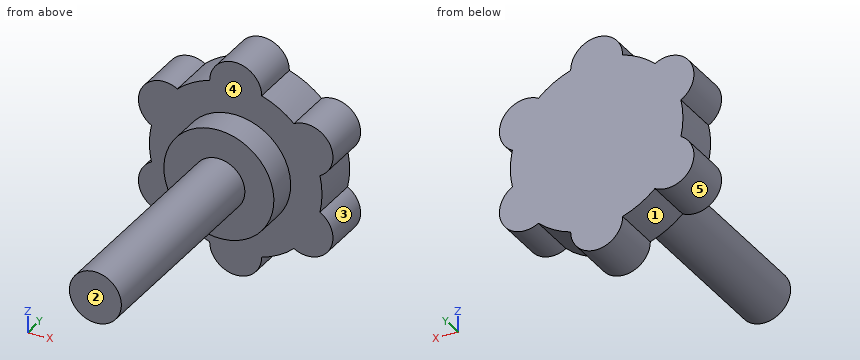
```python
from build123d import *

# Parameters (mm, degrees)
BOSS_EXTRUDE1_DEPTH = 5.6
SKETCH2_R           = 6.35
BOSS_EXTRUDE2_DEPTH = 3.4
SKETCH3_R           = 3
BOSS_EXTRUDE3_DEPTH = 25


with BuildPart() as part:
    # Sketch1 → Boss-Extrude1 (new body)
    with BuildSketch(Plane(origin=(0, 0, 0), x_dir=(1, 0, 0), z_dir=(0, 1, 0))):
        with BuildLine():
            Line((-9.72424134, -2.15192377), (-9.725740285, -2.152789186))
            ThreePointArc((-9.725740285, -2.152789186), (-10.823817926, -6.250865027), (-6.725742085, -7.348942669))
            Line((-6.725742085, -7.348942669), (-6.723420775, -7.34760246))
            ThreePointArc((-6.723420775, -7.34760246), (-4.978167749, -8.626268935), (-2.998, -9.497952231))
            Line((-2.998, -9.497952231), (-2.998, -9.5))
            ThreePointArc((-2.998, -9.5), (0.002000003, -12.499999996), (3.002, -9.499999993))
            Line((3.002, -9.499999993), (3.002, -9.497636397))
            ThreePointArc((3.002, -9.497636397), (4.982303032, -8.625613539), (6.727581168, -7.346540363))
            Line((6.727581168, -7.346540363), (6.728741336, -7.347210186))
            ThreePointArc((6.728741336, -7.347210186), (10.826817547, -6.249133975), (9.728741336, -2.151057763))
            Line((9.728741336, -2.151057763), (9.727581168, -2.15038794))
            ThreePointArc((9.727581168, -2.15038794), (9.962651964, 0.001128196), (9.727467916, 2.152631955))
            ThreePointArc((9.727467916, 2.152631955), (10.825817547, 6.250866025), (6.727194396, 7.348626461))
            ThreePointArc((6.727194396, 7.348626461), (4.981167779, 8.628000969), (3, 9.5))
            ThreePointArc((3, 9.5), (2e-09, 12.5), (-3, 9.499052498))
            ThreePointArc((-3, 9.499052498), (-4.980665222, 8.626558938), (-6.726128008, 7.346856081))
            ThreePointArc((-6.726128008, 7.346856081), (-10.824817547, 6.249133975), (-9.726741336, 2.151057764))
            Line((-9.726741336, 2.151057764), (-9.725033927, 2.150071991))
            ThreePointArc((-9.725033927, 2.150071991), (-9.959651798, -0.000969188), (-9.72424134, -2.15192377))
        make_face()
    extrude(amount=BOSS_EXTRUDE1_DEPTH)

    # Sketch2 → Boss-Extrude2 (add)
    with BuildSketch(Plane.XZ):
        with Locations(Location((0, 0, 0), (0, 0, 90))):
            Circle(SKETCH2_R)
    extrude(amount=BOSS_EXTRUDE2_DEPTH)

    # Sketch3 → Boss-Extrude3 (add)
    with BuildSketch(Plane.XZ.offset(3.4)):
        with Locations(Location((0, 0, 0), (0, 0, 270))):
            Circle(SKETCH3_R)
    extrude(amount=BOSS_EXTRUDE3_DEPTH)


solid = part.part
```
Build history of the part. All positions in model axes, mm. Face numbers are marked on the shaded views. A direction names the side the tool comes from. Give positions to 0.01 mm unless a question says otherwise; leave off trailing zeros. Loops run counter-clockwise (first coordinate to the right, second up) from the corner with the lowest first, then second, coordinate; pieces in that order, holes last.
Item 1: Drill centre lines: line 1 (Y direction, x = -5, z = -7.25); line 2 (X direction, y = -2.5, z = -0.25); line 3 (Y direction, x = 1.25, z = 5.25). Where is each one in solid material? Low to high.
Answers follow:
line 1: y = 0 to 5.6
line 2: x = -6.35 to 6.35
line 3: y = -3.4 to 5.6
Item 2: Which spindle directions (+Z, -Z, +X, -X, +Y, -Y) get a long thin tool onto all of the face, cutting with end or side? Do the marked faces 4 and 5. Say none if no direction does.
Answers follow:
face 4: -Y
face 5: +Y, -Y
Item 3: Slice it at A-A, the plane x = 0. List the corners of the cut face in (y, z), and give its area (3 significant figures).
Answers follow:
outline: (-28.4, -3) - (-3.4, -3) - (-3.4, -6.35) - (0, -6.35) - (0, -12.5) - (5.6, -12.5) - (5.6, 12.5) - (0, 12.5) - (0, 6.35) - (-3.4, 6.35) - (-3.4, 3) - (-28.4, 3) - close
area: 333 mm2
Item 4: Flat gauge pins, fed straight in: pin 1 (2 mm diameter, centred on y = -3, z = -1, fed in from -X); pin 2 (10 mm diameter, centred on y = -2, z = -0.5, fed in from +X); pin 3 (3 mm diameter, centred on x = -8.5, z = -2, fed in from -Y); pin 4 (2 mm diameter, centred on x = 6, z = 1.5, fed in from -Y). Where does each tip first touch, or does it go through?
Answers follow:
pin 1: stops at x = -6.35
pin 2: stops at x = 11.23
pin 3: stops at y = 0
pin 4: stops at y = -3.4
Item 5: Pull direction Z, two halves, no side cores. Call the marked faces 1, 2 and 3: released by +Z, released by -Z, zero draft, split by the parting line, or undercut.
Answers follow:
face 1: released by -Z
face 2: zero draft
face 3: undercut
Item 6: Slice it at B-B, the plane z = 0. List the corners of the cut face in (x, y).
Answers follow:
outline: (-9.96, 0) - (-6.35, 0) - (-6.35, -3.4) - (-3, -3.4) - (-3, -28.4) - (3, -28.4) - (3, -3.4) - (6.35, -3.4) - (6.35, 0) - (9.96, 0) - (9.96, 5.6) - (-9.96, 5.6) - close
Item 7: Slice it at D-D, the plane z = 5.75. List the corners of the cut face in (x, y).
Answers follow:
outline: (-11.05, 0) - (-2.69, 0) - (-2.69, -3.4) - (2.69, -3.4) - (2.69, 0) - (11.06, 0) - (11.06, 5.6) - (-11.05, 5.6) - close
